Check sheet for the modelled part. Datum: model origin and axes. Units: mm. Face numbers are marked on the shaded views. Round coordinates to 2 decimals unless told otherwise and drop trailing zeros. Write each loop counter-clockwise with the first axis right and the second up, starting at its lowest first coordinate (ties: lowest second). Pieces come first, ordered by that corner, then holes.
Item 1: Depth check by flat-ended pin: pin 1 (3 mm diameter, centred on x = 0.5, z = 1.5, fed in from -Y); pin 2 (4 mm diameter, centred on x = 2.5, y = 2, fed in from -Z); pin 3 (0.8 mm diameter, centred on x = 0, z = 0, fed in from +Y). Enter the tip coordinate at first touch or a pass-through.
Item 2: Section check C-C, the plane y = 11. Record the cut outline in (x, z), plus the area to 3 significant figures.
Item 3: Material ranges on line 1 along X through (y, z) = (3.75, 0); line 2 along X through (y, z) = (8, 0); line 3 along Y through (x, z) = (-1.5, -2.25), recorded low to high.
Item 4: Release check for a two-part mould opening along Z. For the marked faces 1, 2 and 3 record: pulls with the +Z half, pulls with the -Z half, needs draft (parallel to the pull), parting line crosses it, or undercut.
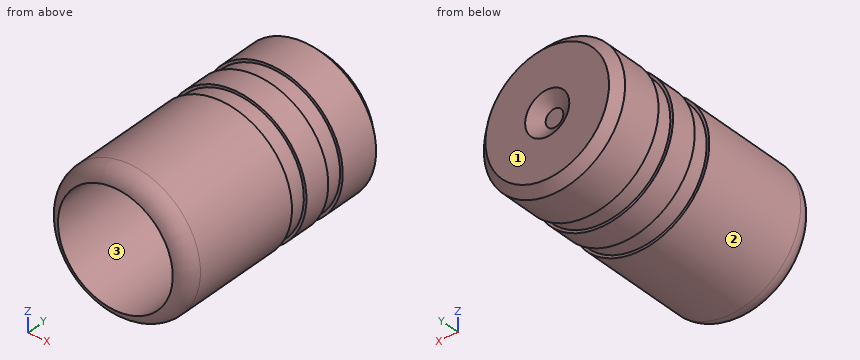
from build123d import *


with BuildPart() as part:
    # 草图1 → 旋转1 (revolve)
    with BuildSketch(Plane.XY, mode=Mode.PRIVATE) as revolve_1_sk:
        with BuildLine():
            Line((-3.25, 0), (-3.25, 12.5))
            Line((-3.25, 12.5), (0, 12.5))
            Line((0, 12.5), (0, 13.1))
            Line((0, 13.1), (-0.5, 13.1))
            Line((-0.5, 13.1), (-1.25, 13.6))
            Line((-1.25, 13.6), (-3.5, 13.6))
            Line((-3.5, 13.6), (-4, 13.1))
            Line((-4, 13.1), (-4, 10.8))
            Line((-4, 10.8), (-3.85, 10.8))
            Line((-3.85, 10.8), (-3.85, 9.8))
            Line((-3.85, 9.8), (-4, 9.8))
            Line((-4, 9.8), (-4, 8.3))
            Line((-4, 8.3), (-3.85, 8.3))
            Line((-3.85, 8.3), (-3.85, 7.3))
            Line((-3.85, 7.3), (-4, 7.3))
            Line((-4, 7.3), (-4, 1))
            ThreePointArc((-4, 1), (-3.791666667, 0.375), (-3.25, 0))
        make_face()
    revolve(revolve_1_sk.sketch.rotate(Axis((0, 0, 0), (0, 1, 0)), 270), axis=Axis((0, 0, 0), (0, 1, 0)))


solid = part.part
Values found:
1. pin 1: stops at y = 12.5
1. pin 2: stops at z = -3.97
1. pin 3: stops at y = 13.1
2. outline: circle Ø8 at (0, 0); hole circle Ø6.5 at (0, 0)
2. area: 17.1 mm2
3. line 1: x = -4 to -3.25, 3.25 to 4
3. line 2: x = -3.85 to -3.25, 3.25 to 3.85
3. line 3: y = 12.5 to 13.6
4. face 1: needs draft
4. face 2: parting line crosses it
4. face 3: undercut
